from build123d import *

# Parameters (mm, degrees)
EXTRUDE_642_DEPTH   = 1648
SKETCH_2_W          = 64
SKETCH_2_H          = 64
EXTRUDE_1_DEPTH     = 85
SKETCH_4_W          = 54
SKETCH_4_H          = 12
EXTRUDE_2_DEPTH     = 10
CUT_EXTRUDE_1_DEPTH = 10
SKETCH_6_W          = 64
SKETCH_6_H          = 69
EXTRUDE_3_DEPTH     = 15
SKETCH_7_W          = 48
SKETCH_7_H          = 88
EXTRUDE_4_DEPTH     = 88
SKETCH_8_R          = 36.5
CUT_EXTRUDE_2_DEPTH = 3
SKETCH_9_R          = 8
EXTRUDE_5_DEPTH     = 19


with BuildPart() as part:
    # 草图1 → Extrude 642 (new body)
    with BuildSketch(Plane.XY):
        Polygon((9.931917842, 6.925864063), (9.931917842, 41.925864063), (12.931917842, 41.925864063), (12.931917842, 40.425864063), (16.931917842, 40.425864063), (16.931917842, 48.425864063), (12.931917842, 48.425864063), (12.931917842, 46.925864063), (9.931917842, 46.925864063), (9.931917842, 56.425864063), (73.931917842, 56.425864063), (73.931917842, 46.925864063), (70.931917842, 46.925864063), (70.931917842, 48.425864063), (66.931917842, 48.425864063), (66.931917842, 40.425864063), (70.931917842, 40.425864063), (70.931917842, 41.925864063), (73.931917842, 41.925864063), (73.931917842, 6.925864063), (70.931917842, 6.925864063), (70.931917842, 8.425864063), (66.931917842, 8.425864063), (66.931917842, 0.425864063), (70.931917842, 0.425864063), (70.931917842, 1.925864063), (73.931917842, 1.925864063), (73.931917842, -7.574135937), (9.931917842, -7.574135937), (9.931917842, 1.925864063), (12.931917842, 1.925864063), (12.931917842, 0.425864063), (16.931917842, 0.425864063), (16.931917842, 8.425864063), (12.931917842, 8.425864063), (12.931917842, 6.925864063), align=None)
    extrude(amount=-EXTRUDE_642_DEPTH)

    # 草图2 → 凸台-拉伸1 (add)
    with BuildSketch(Plane.XY):
        with Locations((41.931917842, 24.425864063)):
            Rectangle(SKETCH_2_W, SKETCH_2_H)
    extrude(amount=EXTRUDE_1_DEPTH)

    # 草图4 → 凸台-拉伸2 (add)
    with BuildSketch(Plane(origin=(0, 56.425864063, 0), x_dir=(-1, 0, 0), z_dir=(0, 1, 0))):
        with Locations((-41.931917842, 6)):
            Rectangle(SKETCH_4_W, SKETCH_4_H)
    extrude(amount=EXTRUDE_2_DEPTH)

    # 草图5 → 切除-拉伸1 (cut)
    with BuildSketch(Plane(origin=(73.931917842, 0, 0), x_dir=(0, 0, -1), z_dir=(1, 0, 0))):
        with BuildLine():
            Line((0, 48.925864063), (-6, 48.925864063))
            ThreePointArc((-6, 48.925864063), (-8.828427125, 47.754291188), (-10, 44.925864063))
            Line((-10, 44.925864063), (-10, 43.925864063))
            ThreePointArc((-10, 43.925864063), (-8.828427125, 41.097436938), (-6, 39.925864063))
            Line((-6, 39.925864063), (0, 39.925864063))
            Line((0, 39.925864063), (0, 48.925864063))
        make_face()
        with BuildLine():
            Line((0, 8.925864063), (-6, 8.925864063))
            ThreePointArc((-6, 8.925864063), (-8.828427125, 7.754291188), (-10, 4.925864063))
            Line((-10, 4.925864063), (-10, 3.925864063))
            ThreePointArc((-10, 3.925864063), (-8.828427125, 1.097436938), (-6, -0.074135937))
            Line((-6, -0.074135937), (0, -0.074135937))
            Line((0, -0.074135937), (0, 8.925864063))
        make_face()
    cut_extrude_1 = extrude(amount=-CUT_EXTRUDE_1_DEPTH, mode=Mode.SUBTRACT)

    # 镜向1: 切除-拉伸1 across plane
    add(cut_extrude_1.mirror(Plane.ZY.offset(-41.931917842)), mode=Mode.SUBTRACT)

    # 草图6 → 凸台-拉伸3 (add)
    with BuildSketch(Plane(origin=(0, 0, -1648), x_dir=(-1, 0, 0), z_dir=(0, 0, -1))):
        with Locations((-41.931917842, 26.925864063)):
            Rectangle(SKETCH_6_W, SKETCH_6_H)
    extrude(amount=EXTRUDE_3_DEPTH)

    # 草图7 → 凸台-拉伸4 (add)
    with BuildSketch(Plane(origin=(0, 0, -1663), x_dir=(-1, 0, 0), z_dir=(0, 0, -1))):
        with Locations((-41.931917842, 24.425864063)):
            Rectangle(SKETCH_7_W, SKETCH_7_H)
    extrude(amount=EXTRUDE_4_DEPTH)

    # 草图8 → 切除-拉伸2 (cut)
    with BuildSketch(Plane.ZY.offset(-17.931917842)):
        with Locations((-1707, 24.425864063)):
            Circle(SKETCH_8_R)
    cut_extrude_2 = extrude(amount=-CUT_EXTRUDE_2_DEPTH, mode=Mode.SUBTRACT)

    # 草图9 → 凸台-拉伸5 (add)
    with BuildSketch(Plane.ZY.offset(-20.931917842)):
        with Locations((-1707, 24.425864063)):
            Circle(SKETCH_9_R)
    extrude_5 = extrude(amount=EXTRUDE_5_DEPTH)

    # 镜向2: 切除-拉伸2, 凸台-拉伸5 across plane
    add(cut_extrude_2.mirror(Plane.ZY.offset(-41.931917842)), mode=Mode.SUBTRACT)
    add(extrude_5.mirror(Plane.ZY.offset(-41.931917842)))


solid = part.part
Verification items for the finished model (mm, model axes). A direction names the side the tool comes from. Coordinates: 2 decimals unless noted, no trailing zeros. Write each loop counter-clockwise with the first axis right and the second up, starting at its lowest first coordinate (ties: lowest second). Pieces come first, ordered by that corner, then holes. Notation, with made-up numbers: M 39,11 L 80,11 A24 ccw 80,42 Z; hole C 73.5,34.25 d10. An arc over 180 degrees is marked long. Use CSV: the item, a comma, the result in double quotes.
Q1. Set-up check for faces 1 (the flat face through (9.932, 26, -777)), 2 (the flat face through (62.932, 25, -1716)), 3 (the cylindrical face through (19.411, 26.031, -1743.465)): record each of +Z, -Z, +X, -X, +Y, -Y from which the full face is reachable in a straight line by a thin tool's end or side.
Computed values:
face 1,"+Z, -X, +Y, -Y"
face 2,"+X"
face 3,"-X"
Q2. Section check A-A, the plane x = 39. Enter the section's corners in (y, z).
Computed values:
outline,"M -19.57,-1751 L 68.43,-1751 L 68.43,-1663 L 61.43,-1663 L 61.43,-1648 L 56.43,-1648 L 56.43,0 L 66.43,0 L 66.43,12 L 56.43,12 L 56.43,85 L -7.57,85 L -7.57,-1663 L -19.57,-1663 Z"
Q3. Thickness scan on line 1 along X through (y, z) = (8, -984); line 2 along Y through (x, z) = (63, -1707); line 3 along Z through (x, y) = (11, 47.5). Record the ranges inside material, lowest first. Write a range as [from, to].
Computed values:
line 1,"[9.93, 12.93], [16.93, 66.93], [70.93, 73.93]"
line 2,"[-19.57, -12.07], [16.43, 32.43], [60.93, 68.43]"
line 3,"[-1663, 0], [9.06, 85]"
Q4. Go/stop test with flat-tipped pins: P1, Ø1.5, axis at y = 36.5, z = -627.5, coming from the +X side; P2, Ø4.5, axis at x = 15, z = -478, coming from the +Y side; P3, Ø3, axis at x = 17.5, y = 59.5, coming from the +Z side. Record where each tip stops, or that it passes through.
Computed values:
P1,"x = 73.93"
P2,"y = 56.43"
P3,"z = 12"
Q5. Mould release check, pull along Y, two halves, no side actions. Record for faces 4 (the flat face through (41, 25, 85)), 5 (the flat face through (42, 68.426, -1706)), 6 (the flat face through (20.932, 25, -1716)), 7 (the flat face through (42, -19.574, -1706)): pulls with the +Y half, pulls with the -Y half, needs draft (parallel to the pull), parting line crosses it, or undercut.
Computed values:
face 4,"needs draft"
face 5,"pulls with the +Y half"
face 6,"undercut"
face 7,"pulls with the -Y half"
